from build123d import *

# Parameters (mm, degrees)
EXTRUDE_1_DEPTH        = 42
HOLE_WIZARD_M6_1_D     = 5
HOLE_WIZARD_M6_1_DEPTH = 8
HOLE_WIZARD_M6_1_TIP   = 1.502151548


with BuildPart() as part:
    # 草图1 → 凸台-拉伸1 (new, symmetric)
    with BuildSketch(Plane.XY):
        Polygon((-11.5, -17.25), (-24, -17.25), (-24, 17.25), (24, 17.25), (24, -17.25), (11.5, -17.25), (11.5, -0.75), (-11.5, -0.75), align=None)
    extrude(amount=EXTRUDE_1_DEPTH, both=True)

    # M6 螺纹孔1
    with Locations(Plane(origin=(0, 17.25, 0), x_dir=(1, 0, 0), z_dir=(0, 1, 0))):
        with Locations((-17.5, 17.5), (17.5, 17.5), (17.5, -17.5), (-17.5, -17.5)):
            Hole(HOLE_WIZARD_M6_1_D / 2, depth=HOLE_WIZARD_M6_1_DEPTH)
            with Locations((0, 0, -(HOLE_WIZARD_M6_1_DEPTH + HOLE_WIZARD_M6_1_TIP / 2))):  # 118° drill point
                Cone(0, HOLE_WIZARD_M6_1_D / 2, HOLE_WIZARD_M6_1_TIP, mode=Mode.SUBTRACT)


solid = part.part
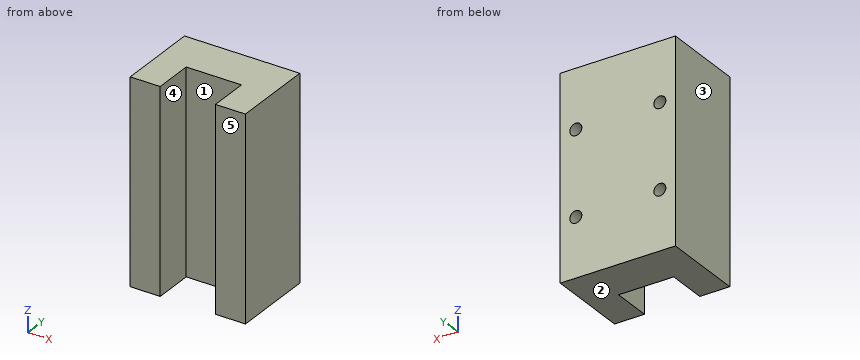
Work out the finished part from the listing and answer in its coordinate system (mm). Face numbers are marked on the shaded views. A direction names the side the tool comes from. Give positions to 0.01 mm unless a question says otherwise; leave off trailing zeros. Order: outer loops, then holes, each group sorted by start corner. A loop starts at its lowest first (then second) coordinate and runs counter-clockwise, first axis right, second up. Notation, with made-up numbers: (-1.75, -13) -> (8.25, -13) arc R19 ccw to (8.25, 20) -> close; hole circle Ø6 at (68.25, 50.25). An arc over 180 degrees is marked (long way). Answer as a JSON object with one key per item and string values. Group by question number.
1. Section A-A on y = -10.5 is taken. Determine the outline of the cut face in (x, z).
2. The mould has two halves that part along X. Classify the marked faces 1, 2 and 3: released by +X, released by -X, zero draft, split by the parting line, or undercut.
3. Flat-ended cylindrical pins translate along their axes: pin 1 Ø11.5 at (x, z) = (4.5, -4) entering from -Y; pin 2 Ø4 at (x, z) = (-17.5, -17.5) entering from +Y; pin 3 Ø3 at (x, z) = (-17.5, 17.5) entering from +Y. Find the tip coordinate at first contact, or state that the pin passes through.
4. A tool of negligible diameter and unlimited length cuts with its end or side. For the marked faces 4 and 5, from which of +Z, -Z, +X, -X, +Y, -Y can it reach the whole face along a straight path? Write none if from no direction.
5. Section C-C on x = 0 is taken. Determine the outline of the cut face in (y, z), plus the area to 3 significant figures.
6. Section B-B on z = -33.5 is taken. Determine the outline of the cut face in (x, y).
7. Consider line 1 along Z through (x, y) = (17.5, 13.25); line 2 along X through (y, z) = (13.5, 17.5); line 3 along Z through (x, y) = (-17, 11). Determine where each line is inside the solid, lowest interval first. Write a range as [from, to].
Result sheet:
{
 "1": {"outline": "(-24, -42) -> (-11.5, -42) -> (-11.5, 42) -> (-24, 42) -> close; (11.5, -42) -> (24, -42) -> (24, 42) -> (11.5, 42) -> close"},
 "2": {"face 1": "undercut", "face 2": "zero draft", "face 3": "released by -X"},
 "3": {"pin 1": "stops at y = -0.75", "pin 2": "stops at y = 8.95", "pin 3": "stops at y = 8.65"},
 "4": {"face 4": "+Z, -Z, -Y", "face 5": "+Z, -Z, +X, -X, -Y"},
 "5": {"outline": "(-0.75, -42) -> (17.25, -42) -> (17.25, 42) -> (-0.75, 42) -> close", "area": "1,510 mm^2"},
 "6": {"outline": "(-24, -17.25) -> (-11.5, -17.25) -> (-11.5, -0.75) -> (11.5, -0.75) -> (11.5, -17.25) -> (24, -17.25) -> (24, 17.25) -> (-24, 17.25) -> close"},
 "7": {"line 1": "z = [-42, -20], [-15, 15], [20, 42]", "line 2": "x = [-24, -20], [-15, 15], [20, 24]", "line 3": "z = [-42, -19.95], [-15.05, 15.05], [19.95, 42]"}
}
